Check sheet for the drawn part. Datum: minimum x, y, z corner. Units: mm. Give positions to 0.01 mm unless a question says otherwise; leave off trailing zeros. Order: outer loops, then holes, each group sorted by start corner. A loop starts at its lowest first (then second) coordinate and runs counter-clockwise, first axis right, second up.
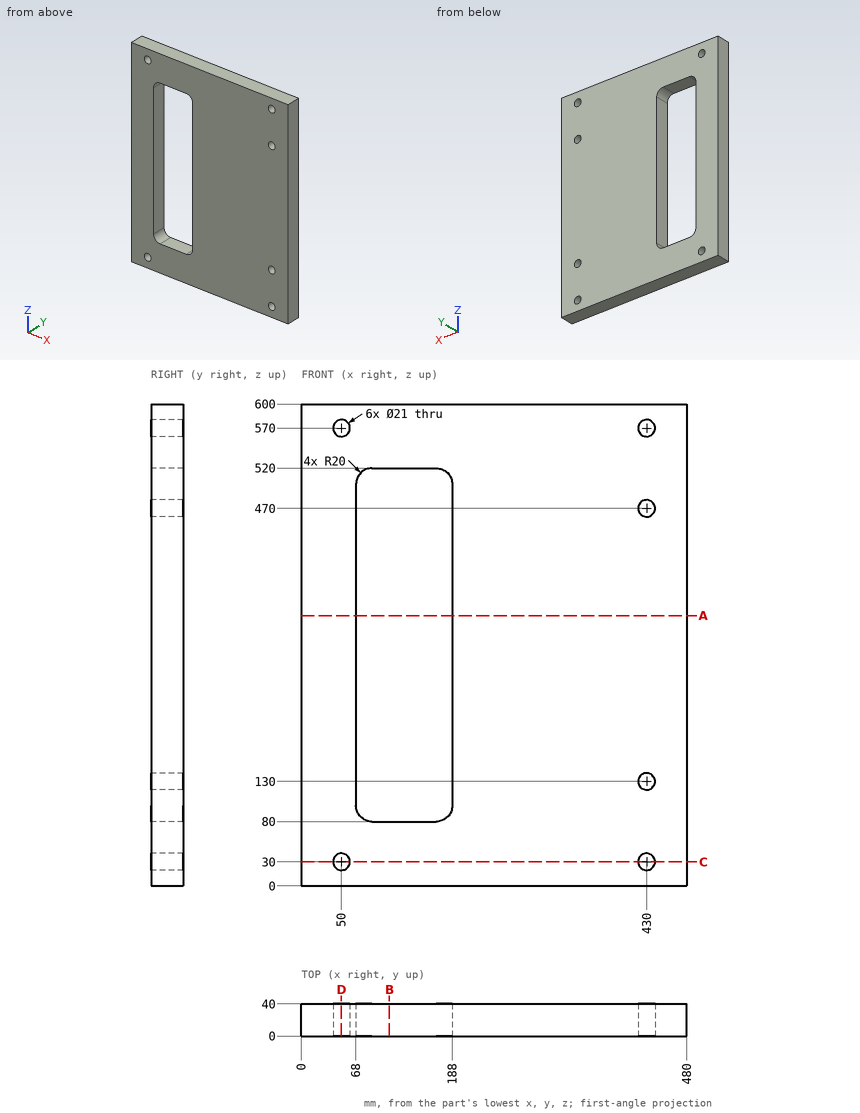
Item 1: Sectioned sample at D-D (x = 50). Enter the section's corners in (y, z).
Reported:
outline: (0, 0) - (40, 0) - (40, 19.5) - (0, 19.5) - close; (0, 40.5) - (40, 40.5) - (40, 559.5) - (0, 559.5) - close; (0, 580.5) - (40, 580.5) - (40, 600) - (0, 600) - close
Item 2: Sectioned sample at B-B (x = 109.5). Enter the section's corners in (y, z), and give its area (3 significant figures).
Reported:
outline: (0, 0) - (40, 0) - (40, 80) - (0, 80) - close; (0, 520) - (40, 520) - (40, 600) - (0, 600) - close
area: 6,400 mm2
Item 3: Gauge pin test, flat end, axial feed: pin 1 (20 mm diameter, centred on y = 26, z = 235.5, fed in from -X). Record the tip position at first contact, or that the pin passes through.
Reported:
pin 1: stops at x = 0
Item 4: Sectioned sample at A-A (z = 336.5). Enter the section's corners in (x, y).
Reported:
outline: (0, 0) - (68, 0) - (68, 40) - (0, 40) - close; (188, 0) - (480, 0) - (480, 40) - (188, 40) - close
Item 5: Sectioned sample at C-C (z = 30). Enter the section's corners in (x, y), and give its area (3 significant figures).
Reported:
outline: (0, 0) - (39.5, 0) - (39.5, 40) - (0, 40) - close; (60.5, 0) - (419.5, 0) - (419.5, 40) - (60.5, 40) - close; (440.5, 0) - (480, 0) - (480, 40) - (440.5, 40) - close
area: 17,500 mm2
Item 6: Scan lines: L1, parallel to X at y = 19, z = 30; L2, parallel to Z at x = 429.5, y = 37.5; L3, parallel to Z at x = 50, y = 15. Record each from-to range of solid material in increasing order.
Reported:
L1: x = 0 to 39.5, 60.5 to 419.5, 440.5 to 480
L2: z = 0 to 19.51, 40.49 to 119.51, 140.49 to 459.51, 480.49 to 559.51, 580.49 to 600
L3: z = 0 to 19.5, 40.5 to 559.5, 580.5 to 600
